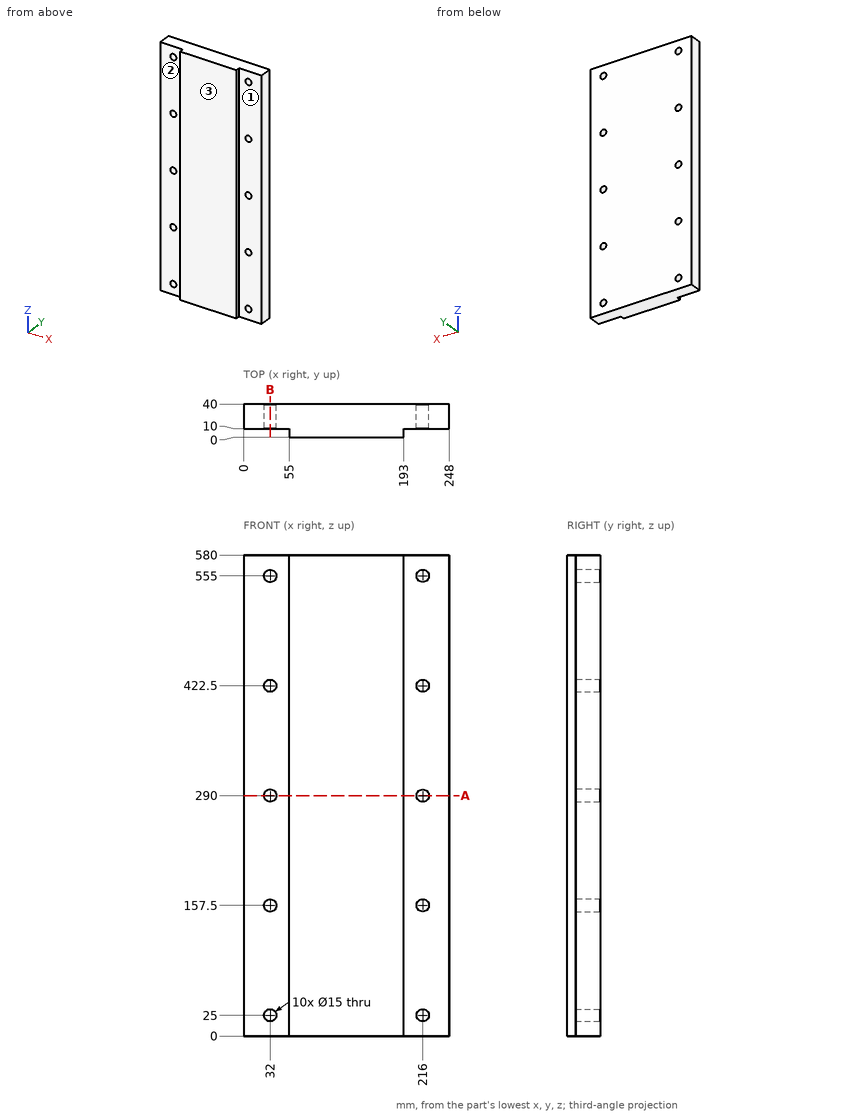
Design review of the part shown in the three views and the two pictorial views. Dimensions are in mm from the part's minimum x, y and z. A direction names the side the tool comes from. Round coordinates to 2 decimals unless told otherwise and drop trailing zeros. Loops run counter-clockwise (first coordinate to the right, second up) from the corner with the lowest first, then second, coordinate; pieces in that order, holes last.
Q1. Machinability: for the marked faces 1, 2 and 3, which of the approach directions +Z, -Z, +X, -X, +Y, -Y give a long, thin tool a straight path to every point of the face, cutting with its end or side? Answer none if there is none.
Result sheet:
face 1: +Z, -Z, +X, -Y
face 2: +Z, -Z, -X, -Y
face 3: +Z, -Z, +X, -X, -Y
Q2. To check wall thickness, follow line 1 along X through (y, z) = (22, 422); line 2 along Z through (x, y) = (32, 34); line 3 along Y through (x, z) = (36.5, 493). State the ranges of each line that lie inside material, in increasing order.
Result sheet:
line 1: x = 0 to 24.52, 39.48 to 208.52, 223.48 to 248
line 2: z = 0 to 17.5, 32.5 to 150, 165 to 282.5, 297.5 to 415, 430 to 547.5, 562.5 to 580
line 3: y = 10 to 40
Q3. Insertion check: pin 1 Ø24 at (x, z) = (32, 157.5) entering from -Y; pin 2 Ø11 at (y, z) = (3.5, 343) entering from -X; pin 3 Ø5 at (y, z) = (3.5, 279) entering from +X. Each pin has a flat end and moves straight along its axis. Give the tip position at first contact, or say it passes through.
Result sheet:
pin 1: stops at y = 10
pin 2: stops at x = 55
pin 3: stops at x = 193
Q4. Add section A-A on z = 290. Write out the cut boundary in (x, y).
Result sheet:
outline: (0, 10) - (24.5, 10) - (24.5, 40) - (0, 40) - close; (39.5, 10) - (55, 10) - (55, 0) - (193, 0) - (193, 10) - (208.5, 10) - (208.5, 40) - (39.5, 40) - close; (223.5, 10) - (248, 10) - (248, 40) - (223.5, 40) - close
Q5. Add section B-B on x = 32. Write out the cut boundary in (y, z), plus the area to 4 significant figures.
Result sheet:
outline: (10, 0) - (40, 0) - (40, 17.5) - (10, 17.5) - close; (10, 32.5) - (40, 32.5) - (40, 150) - (10, 150) - close; (10, 165) - (40, 165) - (40, 282.5) - (10, 282.5) - close; (10, 297.5) - (40, 297.5) - (40, 415) - (10, 415) - close; (10, 430) - (40, 430) - (40, 547.5) - (10, 547.5) - close; (10, 562.5) - (40, 562.5) - (40, 580) - (10, 580) - close
area: 15,150 mm2
